Could you check a few things on this model? Use its own coordinates, in mm. Round coordinates to 2 decimals unless told otherwise and drop trailing zeros. Write each loop counter-clockwise with the first axis right and the second up, starting at its lowest first coordinate (ties: lowest second). Pieces come first, ordered by that corner, then holes. Notation, with made-up numbers: (47.25, -15) - (79.25, -15) arc R21 ccw to (79.25, -10) - close; hole circle Ø2 at (87, 76.5). An arc over 180 degrees is marked (long way). Put each result on its own line as item: value.
from build123d import *

# Parameters (mm, degrees)
SKETCH11_R          = 2.5
MEMBER_1_DEPTH      = 1386
CUT_EXTRUDE_1_DEPTH = 694.324599304
HOLE_WIZARD_M6_1_D  = 5


with BuildPart() as part:
    # Sketch11 → Member 1 (new body)
    with BuildSketch(Plane(origin=(-693, 0, 0), x_dir=(0, 0, -1), z_dir=(1, 0, 0))):
        with BuildLine():
            Line((-6, -15), (-3.25, -15))
            Line((-3.25, -15), (-3.25, -12.7))
            Line((-3.25, -12.7), (-5, -12.7))
            Line((-5, -12.7), (-5, -7))
            ThreePointArc((-5, -7), (0, -4.31662479), (5, -7))
            Line((5, -7), (5, -12.7))
            Line((5, -12.7), (3.25, -12.7))
            Line((3.25, -12.7), (3.25, -15))
            Line((3.25, -15), (6, -15))
            ThreePointArc((6, -15), (7.060660172, -14.560660172), (7.5, -13.5))
            Line((7.5, -13.5), (7.5, 13.5))
            ThreePointArc((7.5, 13.5), (7.060660172, 14.560660172), (6, 15))
            Line((6, 15), (3.25, 15))
            Line((3.25, 15), (3.25, 12.7))
            Line((3.25, 12.7), (5, 12.7))
            Line((5, 12.7), (5, 7))
            ThreePointArc((5, 7), (0, 4.31662479), (-5, 7))
            Line((-5, 7), (-5, 12.7))
            Line((-5, 12.7), (-3.25, 12.7))
            Line((-3.25, 12.7), (-3.25, 15))
            Line((-3.25, 15), (-6, 15))
            ThreePointArc((-6, 15), (-7.060660172, 14.560660172), (-7.5, 13.5))
            Line((-7.5, 13.5), (-7.5, -13.5))
            ThreePointArc((-7.5, -13.5), (-7.060660172, -14.560660172), (-6, -15))
        make_face()
        Circle(SKETCH11_R, mode=Mode.SUBTRACT)
    extrude(amount=MEMBER_1_DEPTH)

    # 草图4 → 切除-拉伸1 (cut, through all)
    with BuildSketch(Plane.XY.offset(7.5)):
        Polygon((-693, 15), (-663, -15), (-693, -15), align=None)
        Polygon((693, -15), (693, 15), (663, -15), align=None)
    extrude(amount=-CUT_EXTRUDE_1_DEPTH, mode=Mode.SUBTRACT)

    # M6 螺纹孔1 (through all)
    with Locations(Plane.XY.offset(7.5)):
        with Locations((-45, 0), (45, 0)):
            Hole(HOLE_WIZARD_M6_1_D / 2)


solid = part.part
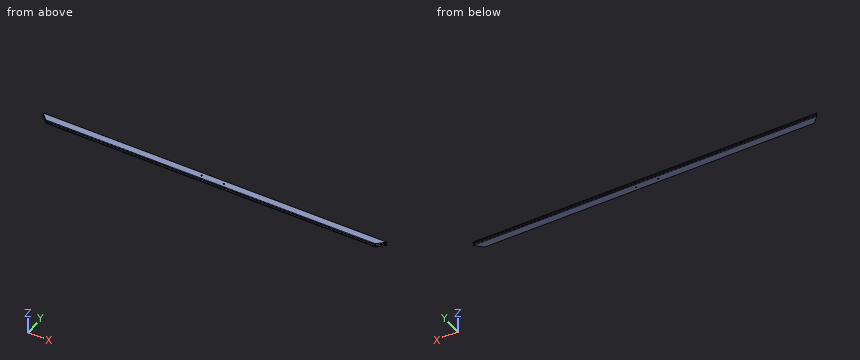
(1) Please list where these lines run through material, in increasing order: probe 1 along Z at (x, y) = (559.5, 8); probe 2 along Z at (x, y) = (-23.5, 0); probe 3 along Y at (x, z) = (-45, -4). Write a range as from..to.
Values found:
probe 1: z = -7.5..-5, 5..7.5
probe 2: z = -7.5..-2.5, 2.5..7.5
probe 3: y = -15..-12.7, -5.84..-2.5, 2.5..5.84, 12.7..15
(2) Imagine slicing it at A-A, the plane x = 509. List the corners of the cut face in (y, z) for me.
Values found:
outline: (-15, -6) arc R1.5 ccw to (-13.5, -7.5) - (13.5, -7.5) arc R1.5 ccw to (15, -6) - (15, -3.25) - (12.7, -3.25) - (12.7, -5) - (7, -5) arc R6 cw to (7, 5) - (12.7, 5) - (12.7, 3.25) - (15, 3.25) - (15, 6) arc R1.5 ccw to (13.5, 7.5) - (-13.5, 7.5) arc R1.5 ccw to (-15, 6) - (-15, 3.25) - (-12.7, 3.25) - (-12.7, 5) - (-7, 5) arc R6 cw to (-7, -5) - (-12.7, -5) - (-12.7, -3.25) - (-15, -3.25) - close; hole circle Ø5 at (0, 0)
(3) I'm going to push flat-ended pins straight in: pin 1 (1 mm diameter, centred on y = 2.5, z = 0, fed in from -X); pin 2 (8 mm diameter, centred on y = 0, z = 0, fed in from -X); pin 3 (4 mm diameter, centred on y = 0, z = 5, fed in from +X). Where does each tip first touch, or does it pass through?
Values found:
pin 1: stops at x = -681
pin 2: stops at x = -682
pin 3: stops at x = 680
